from build123d import *

# Parameters (mm, degrees)
CUT_EXTRUDE1_DEPTH      = 27.896141003
CUT_EXTRUDE1_DEPTH_BACK = 27.896141003


with BuildPart() as part:
    # Sweep2: sweep along a path in Dimension sketch
    with BuildLine(Plane.XY) as sweep2_path:
        Line((23.5, 1.45), (3.5, 1.45))
        ThreePointArc((3.5, 1.45), (2.715712277, 1.606029633), (2.050862219, 2.050357081))
        ThreePointArc((2.050862219, 2.050357081), (-2.9, 0), (2.050862219, -2.050357081))
        ThreePointArc((2.050862219, -2.050357081), (2.715712277, -1.606029633), (3.5, -1.45))
        Line((3.5, -1.45), (26.7, -1.45))
    # Sketch2 → Sweep2 (sweep)
    with BuildSketch(Plane(origin=(23.5, 1.45, 0), x_dir=(0, 0, 1), z_dir=(-1, 0, 0))):
        with BuildLine():
            Line((-1.449965517, -1.44), (1.449965517, -1.44))
            ThreePointArc((1.449965517, -1.44), (0, 0), (-1.449965517, -1.44))
        make_face()
    sweep(path=sweep2_path.line)

    # Sketch3 → Cut-Extrude1 (cut, two sides: drawn at the far end of the back side and taken through both)
    with BuildSketch(Plane.XY.offset(-CUT_EXTRUDE1_DEPTH_BACK)):
        Polygon((23.5, 0.72), (22.468093733, 1.45), (26.71, 1.45), (26.71, -1.45), (25.661091657, -1.45), (26.7, -0.73), (25.668093733, 0), (22.461091657, 0), align=None)
    extrude(amount=CUT_EXTRUDE1_DEPTH + CUT_EXTRUDE1_DEPTH_BACK, mode=Mode.SUBTRACT)


solid = part.part
Source: CAD feature listing. Evaluate the final solid. Frame: model axes, mm. A direction names the side the tool comes from. Give positions to 0.01 mm unless a question says otherwise; leave off trailing zeros. Order: outer loops, then holes, each group sorted by start corner. A loop starts at its lowest first (then second) coordinate and runs counter-clockwise, first axis right, second up. Notation, with made-up numbers: (34, 42) -> (74, 42) arc R15 ccw to (74, 63) -> close; hole circle Ø5 at (6.5, -3). An arc over 180 degrees is marked (long way). Use a Markdown table: item, result.
1) Contact query for flat-ended pins moving along their axis: P1, Ø1.5, axis at x = 7.5, z = 0.5, coming from the -Y side; P2, Ø1.4, axis at x = 18.5, z = -0.5, coming from the +Y side. Output: stop coordinate, or through.
Answer list:
| item | result |
|---|---|
| P1 | y = -1.45 |
| P2 | y = 1.45 |
2) Ray query, line 1 along Y through (x, z) = (0, 0); line 2 along Y through (x, z) = (0, -0.5); line 3 along Z through (x, y) = (14.5, -0.9). Return the intervals inside material, ascending. Write a range as [from, to].
Answer list:
| item | result |
|---|---|
| line 1 | [-2.9, -1.46], [1.46, 2.9] |
| line 2 | [-2.81, -1.46], [1.46, 2.81] |
| line 3 | [-1.14, 1.14] |
3) Reachability of faces 1 (the cylindrical face through (2.15, -0.28, 0.02)), 2 (the cylindrical face through (15.26, -1.45, 0.03)), 3 (the flat face through (22.98, 0.36, -0.02)) from +Z, -Z, +X, -X, +Y, -Y: full face, straight path, thin tool, end or side. Return the list, or none.
Answer list:
| item | result |
|---|---|
| face 1 | +Z, -Z |
| face 2 | +X, -Y |
| face 3 | +Z, -Z, +X |
4) Section query A-A, the plane x = 9. Return the cut outline in (y, z).
Answer list:
| item | result |
|---|---|
| outline | (-0.01, -1.45) -> (-0.01, 1.45) arc R1.45 ccw to start; (0.01, -1.45) arc R1.45 ccw to (0.01, 1.45) -> close |
5) Mould query, pull axis X, two halves, no side actions, for faces 4 (the flat face through (26.289, -1.015, -0.018)), 5 (the cylindrical face through (2.18, 0.27, 0.02)), 6 (the cylindrical face through (13.36, 1.45, 0.03)). Classes: +X half, -X half, draft (parallel to the pull), parting line (faces both ways), or undercut.
Answer list:
| item | result |
|---|---|
| face 4 | +X half |
| face 5 | undercut |
| face 6 | draft |
